```python
from build123d import *

# Parameters (mm, degrees)
SKETCH_1_R      = 2
SKETCH_1_R_2    = 19
SKETCH_1_R_3    = 3.91899873
SKETCH_1_R_4    = 3
EXTRUDE_3_DEPTH = 10


with BuildPart() as part:
    # 草图1 → 凸台-拉伸3 (new body)
    with BuildSketch(Plane.XY):
        with BuildLine():
            Line((-14, 128), (-6, 0))
            ThreePointArc((-6, 0), (0, -6), (6, 0))
            add(Edge.make_bspline(
                [(6, 0), (1.588652615, 45.680929706), (5.604102499, 79.643200211), (28.004797731, 112.13093391)],
                knots=[0, 0, 0, 0, 0.788155359, 0.788155359, 0.788155359, 0.788155359], degree=3))
            ThreePointArc((28.004797731, 112.13093391), (50.113637924, 128.900750568), (77, 135.767416406))
            ThreePointArc((77, 135.767416406), (157.787149523, 170.485384951), (196.379869136, 249.494896157))
            ThreePointArc((196.379869136, 249.494896157), (200.439238403, 252.311917913), (202, 257))
            Line((202, 257), (202, 262))
            ThreePointArc((202, 262), (194.5, 269.5), (187, 262))
            ThreePointArc((187, 262), (154.781745931, 184.218254069), (77, 152))
            Line((77, 152), (10, 152))
            ThreePointArc((10, 152), (-6.970562748, 144.970562748), (-14, 128))
        make_face()
        Circle(SKETCH_1_R, mode=Mode.SUBTRACT)
        with Locations((10, 128)):
            Circle(SKETCH_1_R_2, mode=Mode.SUBTRACT)
        with Locations((194.5, 262)):
            Circle(SKETCH_1_R_3, mode=Mode.SUBTRACT)
        with Locations((0, 22)):
            Circle(SKETCH_1_R_4, mode=Mode.SUBTRACT)
    extrude(amount=EXTRUDE_3_DEPTH)


solid = part.part
```
Read the model definition and answer for the solid it produces. Units are mm, in the model's axes. Give positions to 0.01 mm unless a question says otherwise; leave off trailing zeros. Loops run counter-clockwise (first coordinate to the right, second up) from the corner with the lowest first, then second, coordinate; pieces in that order, holes last.
Item 1: The part is cut by section C-C (x = 85). Write down the section's boundary in (y, z), and give its area (3 significant figures).
Item 2: The mould has two halves that part along Y. Classify faces 1 (the cylindrical face through (-0.65, 19.07, 4.93)), 2 (the flat face through (69, 143, 0)), 3 (the flat face through (44, 152, 5)): released by +Y, released by -Y, zero draft, split by the parting line, or undercut.
Item 3: Each of these flat-tipped pins is pushed along its axis until it touches: pin 1 Ø4 at (x, z) = (54.5, 1.5) entering from -Y; pin 2 Ø4.5 at (x, y) = (0, 0) entering from -Z; pin 3 Ø3 at (x, z) = (78, 9) entering from -Y; pin 4 Ø1.5 at (y, z) = (217, 6.5) entering from -X. Where does it stop, or does it pass through?
Item 4: The part is cut by section A-A (y = 142). Write down the section's boundary in (x, z), and give its area (3 significant figures).
Item 5: The part is cut by section D-D (y = 243). Write down the section's boundary in (x, z).
Item 6: The part is cut by section B-B (z = 1.75). Give the number of separate pieces and of enclosed holes in the cut face, and give its area (3 significant figures).
Item 7: Find the intervals of material crossed by line 1 along X through (y, z) = (262, 2.5); line 2 along Y through (x, z) = (0, 7); line 3 along X through (y, z) = (126.5, 5.25), in increasing order.
Taken from the geometry:
1. outline: (136.43, 0) - (152.29, 0) - (152.29, 10) - (136.43, 10) - close
1. area: 159 mm2
2. face 1: undercut
2. face 2: zero draft
2. face 3: released by +Y
3. pin 1: stops at y = 130
3. pin 2: stops at z = 0
3. pin 3: stops at y = 135.74
3. pin 4: stops at x = 177.03
4. outline: (-9.49, 0) - (-2.85, 0) - (-2.85, 10) - (-9.49, 10) - close; (22.85, 0) - (110.3, 0) - (110.3, 10) - (22.85, 10) - close
4. area: 941 mm2
5. outline: (185.35, 0) - (195.56, 0) - (195.56, 10) - (185.35, 10) - close
6. separate pieces: 1
6. enclosed holes: 4
6. area: 6,090 mm2
7. line 1: x = 187 to 190.58, 198.42 to 202
7. line 2: y = -6 to -2, 2 to 19, 25 to 111.84, 144.16 to 149.82
7. line 3: x = -13.91 to -8.94, 28.94 to 45.57
